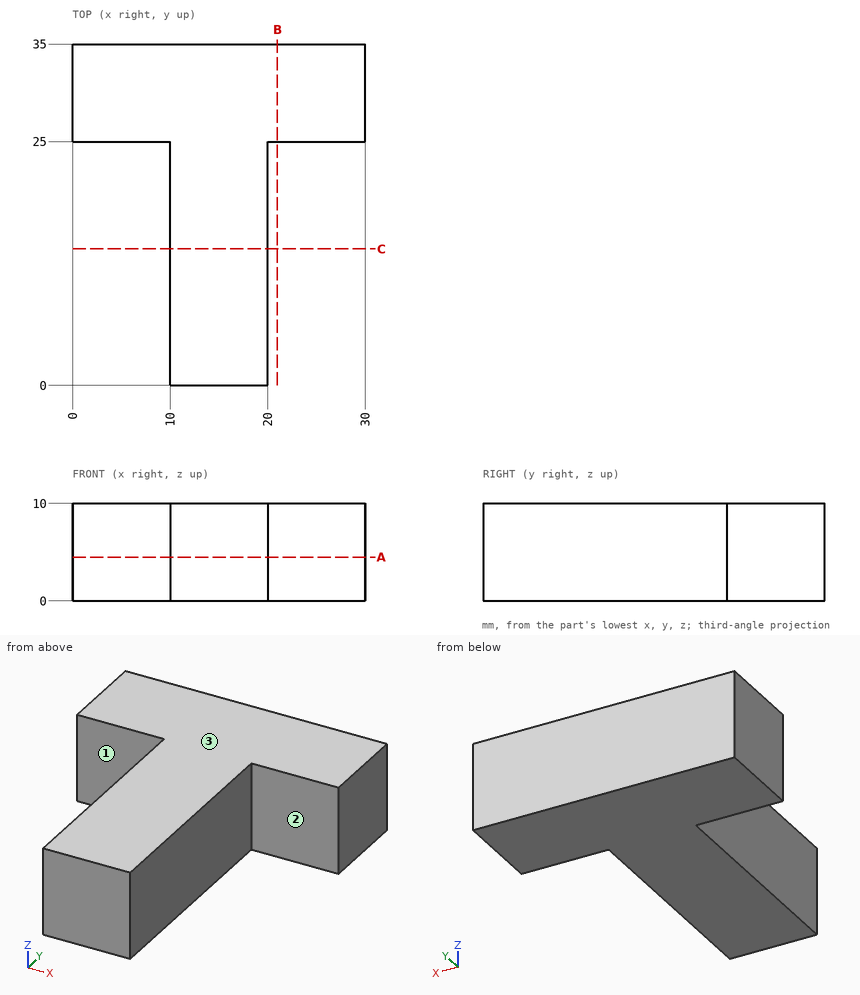
Could you check a few things on this drawing? It's one solid part, dimensions in mm from its lowest x, y, z. A direction names the side the tool comes from. Round coordinates to 2 decimals unless told otherwise and drop trailing zeros. Order: outer loops, then holes, each group sorted by start corner. A loop starts at its lowest first (then second) coordinate and runs counter-clockwise, first axis right, second up. Notation, with made-up numbers: M 28,-0.5 L 59,-0.5 A25 cw 59,30.5 Z; hole C 41.25,7.5 d11. An arc over 180 degrees is marked long. Return JSON: item names as keys, results as strings. Group by question number.
1. I'm going to push flat-ended pins straight in: pin 1 Ø3 at (x, z) = (6.5, 7.5) entering from -Y; pin 2 Ø2 at (y, z) = (14.5, 7) entering from +X; pin 3 Ø6 at (y, z) = (23.5, 4.5) entering from +X; pin 4 Ø4 at (y, z) = (16, 1) entering from -X. Where does each tip first touch, or does it pass through?
2. If we section it at A-A on z = 4.5: List the corners of the cut face in (x, y) for me, then the cut area to 3 significant figures.
3. On a 3-axis mill with a long thin cutter (end or side, diameter ignored), from which of +Z, -Z, +X, -X, +Y, -Y can I reach the whole of each face in a straight line? I mean the marked faces 1, 2 and 3. Say none if no direction works.
4. If we section it at B-B on x = 21: List the corners of the cut face in (y, z) for me, then the cut area to 3 significant figures.
5. Please list where these lines run through material, in increasing order: probe 1 along X at (y, z) = (6, 8); probe 2 along Y at (x, z) = (20.5, 1).
6. If we section it at C-C on y = 14: List the corners of the cut face in (x, z) for me, then the cut area to 3 significant figures.
Reply:
{
 "1": {"pin 1": "y = 25", "pin 2": "x = 20", "pin 3": "x = 30", "pin 4": "x = 10"},
 "2": {"outline": "M 0,25 L 10,25 L 10,0 L 20,0 L 20,25 L 30,25 L 30,35 L 0,35 Z", "area": "550 mm^2"},
 "3": {"face 1": "+Z, -Z, -X, -Y", "face 2": "+Z, -Z, +X, -Y", "face 3": "+Z, +X, -X, +Y, -Y"},
 "4": {"outline": "M 25,0 L 35,0 L 35,10 L 25,10 Z", "area": "100 mm^2"},
 "5": {"probe 1": "10 to 20", "probe 2": "25 to 35"},
 "6": {"outline": "M 10,0 L 20,0 L 20,10 L 10,10 Z", "area": "100 mm^2"}
}
